Input: part model. Units: mm. Frame: model coordinates. Give positions to 0.01 mm unless a question says otherwise; leave off trailing zeros. Order: outer loops, then holes, each group sorted by start corner. A loop starts at its lowest first (then second) coordinate and runs counter-clockwise, first axis right, second up. Notation, with made-up numbers: (47.25, 74.25) - (57.25, 74.25) arc R28 cw to (57.25, 101.25) - close; hole circle Ø10 at (44.25, 40.25). An arc over 180 degrees is marked (long way). Answer in a Markdown table with one row per item. Add a question column.
from build123d import *

# Parameters (mm, degrees)
SKETCH_2_R          = 9.5
SKETCH_3_OUTSIDE_W  = 48.11
SKETCH_3_OUTSIDE_H  = 59.263
SKETCH_3_OUTSIDE_R  = 7.5
CUT_EXTRUDE_1_DEPTH = 50
SKETCH_4_OUTSIDE_W  = 48.11
SKETCH_4_OUTSIDE_H  = 81.514
SKETCH_4_OUTSIDE_R  = 7.5
CUT_EXTRUDE_2_DEPTH = 50


with BuildPart() as part:
    # 扫描1: sweep along a path in 草图1
    with BuildLine(Plane.XY) as sweep_1_path:
        Line((0, 0), (50, 0))
        Line((50, 0), (79.885840943, -2.614672282))
        Line((79.885840943, -2.614672282), (129.126228593, -11.297081166))
    # 草图2 → 扫描1 (sweep)
    with BuildSketch(Plane(origin=(0, 0, 0), x_dir=(0, 0, -1), z_dir=(1, 0, 0))):
        Circle(SKETCH_2_R)
    sweep(path=sweep_1_path.line, transition=Transition.RIGHT)

    # 草图3 outside → 切除-拉伸1 (cut)
    with BuildSketch(Plane.ZY):
        with Locations((0, -5.5765)):
            Rectangle(SKETCH_3_OUTSIDE_W, SKETCH_3_OUTSIDE_H)
        Circle(SKETCH_3_OUTSIDE_R, mode=Mode.SUBTRACT)
    extrude(amount=-CUT_EXTRUDE_1_DEPTH, mode=Mode.SUBTRACT)

    # 草图4 outside → 切除-拉伸2 (cut)
    with BuildSketch(Plane(origin=(127.164511036, -22.422534284, 0), x_dir=(0, 0, -1), z_dir=(0.984807753012208, -0.173648177666931, 0))):
        with Locations((0, 5.863)):
            Rectangle(SKETCH_4_OUTSIDE_W, SKETCH_4_OUTSIDE_H)
        with Locations(Location((0, 11.297081166, 0), (0, 0, 90))):
            Circle(SKETCH_4_OUTSIDE_R, mode=Mode.SUBTRACT)
    extrude(amount=-CUT_EXTRUDE_2_DEPTH, mode=Mode.SUBTRACT)


solid = part.part
Q1. Section B-B, the plane x = 40. Return loops of the section in (y, z).
Q2. Contact query for flat-ended pins moving along their axis: P1, Ø3, axis at x = 18, z = -5, coming from the -Y side; P2, Ø1, axis at y = -11.5, z = -1, coming from the +X side; P3, Ø1, axis at y = -13.5, z = -1, coming from the +X side. Output: stop coordinate, or through.
Q3. Line query: probe 1 along X at (y, z) = (-7.25, -2.5); probe 2 along Y at (x, z) = (77.5, -0.5); probe 3 along Y at (x, z) = (21, 5.75). Output: solid intervals per line, ascending.
Q4. Pull-direction query (X, two-part tool) for faces 1 (the cylindrical face through (81.379, 6.766, -0.209)), 2 (the flat face through (50, 5, -6)), 3 (the cylindrical face through (24.65, 0.33, -7.493)), 4 (the flat face through (80.625, 1.577, 6.378)); classes: +X half, -X half, draft (parallel to the pull), parting line (faces both ways), or undercut.
Q5. Section A-A, the plane z = 0. Return loops of the section in (x, y), then the cut area to 3 significant figures.
Q6. Section C-C, the plane z = 4.75. Return loops of the section in (x, y).
Computed:
| question | item | result |
|---|---|---|
| 1 | outline | circle Ø15 at (0, 0) |
| 2 | P1 | stops at y = -6.63 |
| 2 | P2 | stops at x = 129.18 |
| 2 | P3 | stops at x = 128.83 |
| 3 | probe 1 | x = 50 to 129.84 |
| 3 | probe 2 | y = -11.93 to 7.12 |
| 3 | probe 3 | y = -4.82 to 4.82 |
| 4 | face 1 | +X half |
| 4 | face 2 | -X half |
| 4 | face 3 | draft |
| 4 | face 4 | undercut |
| 5 | outline | (0, -7.5) - (50, -7.5) - (50, -9.54) - (78.23, -12.01) - (78.58, -10) - (127.82, -18.68) - (130.43, -3.91) - (81.19, 4.77) - (81.54, 6.74) - (81.13, 6.81) - (50.41, 9.5) - (50, 9.5) - (50, 7.5) - (0, 7.5) - close |
| 5 | area | 2,070 mm^2 |
| 6 | outline | (0, -5.8) - (50, -5.8) - (50, -8.26) - (78.45, -10.75) - (78.88, -8.33) - (128.12, -17.01) - (130.13, -5.58) - (80.89, 3.1) - (81.31, 5.49) - (80.96, 5.55) - (50.36, 8.23) - (50, 8.23) - (50, 5.8) - (0, 5.8) - close |
